The drawing under review shows one solid part. Ordinate dimensions are in mm from its lowest x, y, z. Coordinates: 2 decimals unless noted, no trailing zeros. Order: outer loops, then holes, each group sorted by start corner. A loop starts at its lowest first (then second) coordinate and runs counter-clockwise, first axis right, second up.
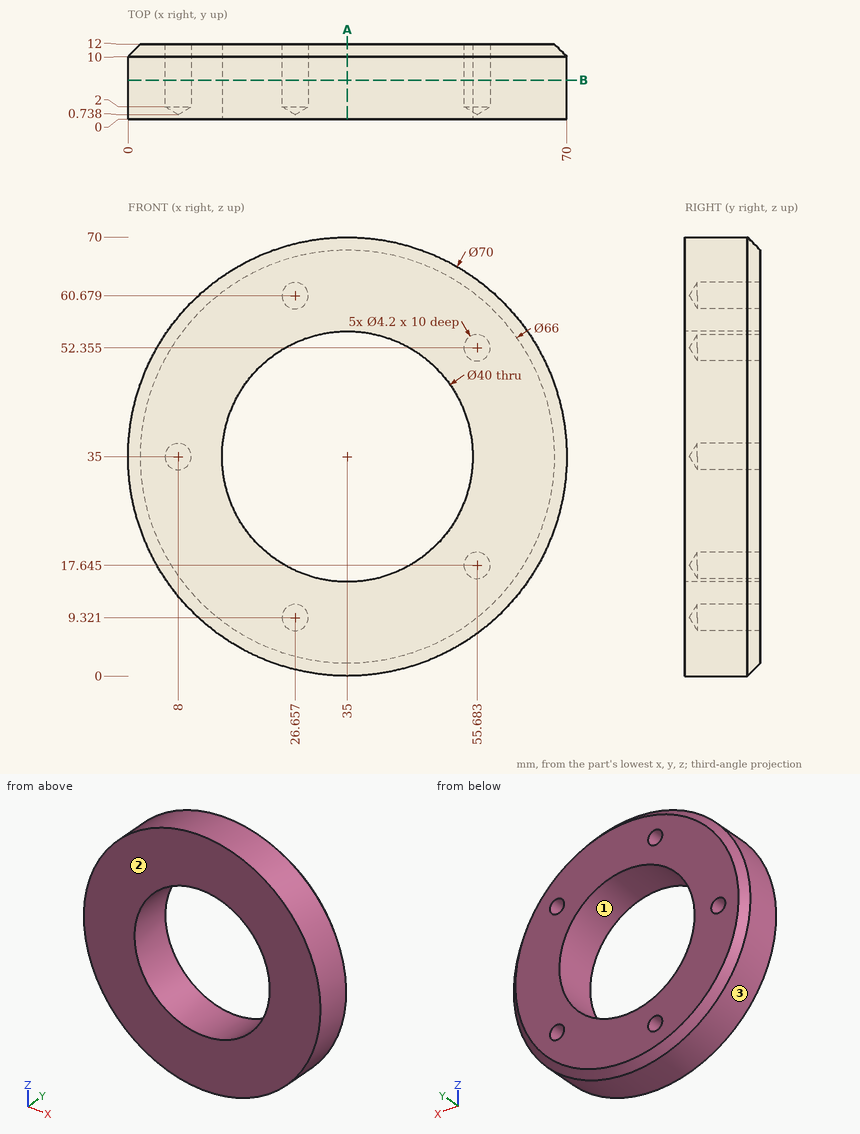
(1) For pin 1 Ø1 at (x, z) = (21, 24) entering from -Y; pin 2 Ø6 at (x, y) = (22, 6.5) entering from -Z; pin 3 Ø1.5 at (x, y) = (22.5, 5.5) entering from -Z; pin 4 Ø1 at (x, y) = (27, 7) entering from +Z, all flat-tipped, find the tip position at first contact; note any pin that passes through.
A:
pin 1: passes through
pin 2: stops at z = 1.46
pin 3: stops at z = 2.03
pin 4: stops at z = 69.19
(2) We need section A-A, the plane x = 35. Write out the cut boundary in (y, z).
A:
outline: (0, 0) - (10, 0) - (12, 2) - (12, 15) - (0, 15) - close; (0, 55) - (12, 55) - (12, 68) - (10, 70) - (0, 70) - close
(3) Draft analysis for pull direction X (two halves, no side actions). For the marked faces 1, 2 and 3, state which applies: released by +X, released by -X, zero draft, split by the parting line, or undercut.
A:
face 1: undercut
face 2: zero draft
face 3: split by the parting line
(4) We need section B-B, the plane y = 6.25. Write out the cut boundary in (x, z) (1 decimal), and give its area (3 significant figures).
A:
outline: circle Ø70 at (35, 35); hole circle Ø4.2 at (8, 35); hole circle Ø40 at (35, 35); hole circle Ø4.2 at (26.7, 9.3); hole circle Ø4.2 at (26.7, 60.7); hole circle Ø4.2 at (55.7, 17.6); hole circle Ø4.2 at (55.7, 52.4)
area: 2,520 mm2
(5) Wall thickness on probe 1 along X at (y, z) = (7.25, 35); probe 2 along X at (y, z) = (3.5, 19) (1 decimal); probe 3 along Z at (x, y) = (50.5, 2.25): over which ranges is each line inside the solid? List them lowest first.
A:
probe 1: x = 0 to 5.9, 10.1 to 15, 55 to 70
probe 2: x = 3.9 to 23, 47 to 54.1, 57.3 to 66.1
probe 3: z = 3.62 to 22.36, 47.64 to 66.38
